Geometry: final body of the model. Coordinates: model frame, mm. A direction names the side the tool comes from. Round coordinates to 2 decimals unless told otherwise and drop trailing zeros. Write each loop counter-clockwise with the first axis right and the second up, starting at its lowest first coordinate (ties: lowest second). Pieces come first, ordered by that corner, then holes. Notation, with made-up numbers: (23, 31.25) -> (31, 31.25) arc R31 cw to (31, 67.25) -> close; hole circle Ø2 at (-4.75, 83). An arc over 180 degrees is marked (long way). One line per item, written item: value. Start each with the question number.
from build123d import *

# Parameters (mm, degrees)
BOSS_EXTRUDE1_DEPTH   = 7.5
SKETCH2_R             = 12
SKETCH2_R_2           = 17.5
SKETCH2_R_3           = 11
SKETCH2_R_4           = 20
SKETCH2_R_5           = 3.4
CUT_EXTRUDE1_DEPTH    = 15
SKETCH3_R             = 3
CUT_EXTRUDE2_DEPTH    = 15
SKETCH4_R             = 3.4
CUT_EXTRUDE3_DEPTH    = 223.514044501
FILLET1_R             = 5
M4_TAPPED_HOLE1_D     = 3.3
M5_TAPPED_HOLE1_D     = 4.2
SKETCH10_W            = 15
SKETCH10_H            = 40
CUT_EXTRUDE4_DEPTH    = 223.892911507
FILLET2_R             = 5
M6_TAPPED_HOLE1_D     = 5
M6_TAPPED_HOLE1_DEPTH = 15
M6_TAPPED_HOLE1_TIP   = 1.502151548


with BuildPart() as part:
    # Sketch1 → Boss-Extrude1 (new, symmetric)
    with BuildSketch(Plane.XY):
        Polygon((207.5, 0), (-207.5, 0), (-207.5, 10), (-192.5, 10), (-192.5, 70), (-207.5, 70), (-207.5, 80), (207.5, 80), (207.5, 70), (192.5, 70), (192.5, 10), (207.5, 10), align=None)
    extrude(amount=BOSS_EXTRUDE1_DEPTH, both=True)

    # Sketch2 → Cut-Extrude1 (cut)
    with BuildSketch(Plane.XY.offset(7.5)):
        with Locations((-142.5, 40)):
            Circle(SKETCH2_R)
        with Locations((9, 40)):
            Circle(SKETCH2_R_2)
        with Locations((72.5, 40)):
            Circle(SKETCH2_R_3)
        with Locations((-79, 40)):
            Circle(SKETCH2_R_4)
        with Locations((142.5, 40)):
            Circle(SKETCH2_R)
        with Locations((-182.5, 40)):
            Circle(SKETCH2_R_5)
        with Locations((182.5, 40)):
            Circle(SKETCH2_R_5)
    extrude(amount=-CUT_EXTRUDE1_DEPTH, mode=Mode.SUBTRACT)

    # Sketch3 → Cut-Extrude2 (cut)
    with BuildSketch(Plane.XY.offset(7.5)):
        with Locations((-35, 69)):
            Circle(SKETCH3_R)
        with Locations((23, 69)):
            Circle(SKETCH3_R)
        with Locations((23, 11)):
            Circle(SKETCH3_R)
        with Locations((-35, 11)):
            Circle(SKETCH3_R)
    extrude(amount=-CUT_EXTRUDE2_DEPTH, mode=Mode.SUBTRACT)

    # Sketch4 → Cut-Extrude3 (cut, through all)
    with BuildSketch(Plane(origin=(0, 80, 0), x_dir=(1, 0, 0), z_dir=(0, 1, 0))):
        with Locations(Location((-202.5, 0, 0), (0, 0, 270))):
            Circle(SKETCH4_R)
        with Locations(Location((202.5, 0, 0), (0, 0, 180))):
            Circle(SKETCH4_R)
    extrude(amount=-CUT_EXTRUDE3_DEPTH, mode=Mode.SUBTRACT)

    # Fillet1
    fillet1_edges = [part.edges().sort_by_distance(p)[0] for p in [
        (-192.5, 10, 0),
        (-192.5, 70, 0),
        (192.5, 70, 0),
        (192.5, 10, 0),
    ]]
    fillet(fillet1_edges, radius=FILLET1_R)

    # M4 Tapped Hole1 (through all)
    with Locations(Plane.XY.offset(7.5)):
        with Locations((47.5, 20), (97.5, 20)):
            Hole(M4_TAPPED_HOLE1_D / 2)

    # M5 Tapped Hole1 (through all)
    with Locations(Plane.XY.offset(7.5)):
        with Locations((-102.55, 63.55), (-55.45, 16.45), (-102.55, 16.45), (-55.45, 63.55)):
            Hole(M5_TAPPED_HOLE1_D / 2)

    # Sketch10 → Cut-Extrude4 (cut, through all)
    with BuildSketch(Plane.XY.offset(7.5)):
        with Locations((-200, 60)):
            Rectangle(SKETCH10_W, SKETCH10_H)
        with Locations((200, 60)):
            Rectangle(SKETCH10_W, SKETCH10_H)
    extrude(amount=-CUT_EXTRUDE4_DEPTH, mode=Mode.SUBTRACT)

    # Fillet2
    fillet2_edges = [part.edges().sort_by_distance(p)[0] for p in [
        (-192.5, 80, 0),
        (192.5, 80, 0),
    ]]
    fillet(fillet2_edges, radius=FILLET2_R)

    # M6 Tapped Hole1
    with Locations(Plane(origin=(0, 0, 0), x_dir=(-1, 0, 0), z_dir=(0, -1, 0))):
        with Locations((-125, 0), (125, 0)):
            Hole(M6_TAPPED_HOLE1_D / 2, depth=M6_TAPPED_HOLE1_DEPTH)
            with Locations((0, 0, -(M6_TAPPED_HOLE1_DEPTH + M6_TAPPED_HOLE1_TIP / 2))):  # 118° drill point
                Cone(0, M6_TAPPED_HOLE1_D / 2, M6_TAPPED_HOLE1_TIP, mode=Mode.SUBTRACT)


solid = part.part
(1) Section query B-B (x = 9). Output: boundary loops of the cut face in (y, z).
(2) Set-up query: faces 5 (the face through (-203.7, 10, 3.4)), 6 (the face through (192.5, 45, 0)), 7 (the face through (207.5, 5, 0)). Return all of +Z, -Z, +X, -X, +Y, -Y with unobstructed straight access to the full face (end or side cutting, diameter ignored); none if empty.
(3) Section query A-A (x = 142.5). Output: boundary loops of the cut face in (y, z), and give its area (3 significant figures).
(4) Line query: probe 1 along X at (y, z) = (36, 6); probe 2 along X at (y, z) = (46, 6.75); probe 3 along Y at (x, z) = (-79, -1.75). Output: solid intervals per line, ascending.
(5) Pin query (flat end, axial travel): pin 1 (2 mm diameter, centred on x = 97.5, y = 20, fed in from +Z); pin 2 (3 mm diameter, centred on y = 61.5, z = 1.5, fed in from -X); pin 3 (8 mm diameter, centred on x = 200, z = 0.5, fed in from +Y); pin 4 (2 mm diameter, centred on y = 17.5, z = 1, fed in from +X). Return the tip coordinate at first contact, or that it passes through.
(6) Pull-direction query (Y, two-part tool) for faces 1 (the face through (205.9, 5.1, 0.1)), 2 (the face through (130.51, 40.53, 0.11)), 3 (the face through (-3, 80, 0)), 4 (the face through (-154.49, 40.53, 0.11)); classes: pulls with the +Y half, pulls with the -Y half, needs draft (parallel to the pull), parting line crosses it, or undercut.
Results list:
1. outline: (0, -7.5) -> (22.5, -7.5) -> (22.5, 7.5) -> (0, 7.5) -> close; (57.5, -7.5) -> (80, -7.5) -> (80, 7.5) -> (57.5, 7.5) -> close
2. face 5: +Z, -Z, -X, +Y
2. face 6: +Z, -Z, +X, +Y
2. face 7: +Z, -Z, +X, +Y, -Y
3. outline: (0, -7.5) -> (28, -7.5) -> (28, 7.5) -> (0, 7.5) -> close; (52, -7.5) -> (80, -7.5) -> (80, 7.5) -> (52, 7.5) -> close
3. area: 840 mm^2
4. probe 1: x = -192.5 to -153.81, -131.19 to -98.6, -59.4 to -8.04, 26.04 to 62.25, 82.75 to 131.19, 153.81 to 192.5
4. probe 2: x = -192.5 to -152.89, -132.11 to -98.08, -59.92 to -7.44, 25.44 to 63.28, 81.72 to 132.11, 152.89 to 192.5
4. probe 3: y = 0 to 20, 60 to 80
5. pin 1: passes through
5. pin 2: stops at x = -192.5
5. pin 3: stops at y = 10.23
5. pin 4: stops at x = 192.5
6. face 1: needs draft
6. face 2: undercut
6. face 3: pulls with the +Y half
6. face 4: undercut
